from build123d import *

# Parameters (mm, degrees)
SKETCH1_W           = 40
SKETCH1_H           = 20
BOSS_EXTRUDE1_DEPTH = 4
M8_TAPPED_HOLE1_D   = 6.8
CUT_EXTRUDE1_DEPTH  = 4
CHAMFER1_SIZE       = 3
CHAMFER2_SIZE       = 0.5


with BuildPart() as part:
    # Sketch1 → Boss-Extrude1 (new body)
    with BuildSketch(Plane.XY):
        Rectangle(SKETCH1_W, SKETCH1_H)
    extrude(amount=BOSS_EXTRUDE1_DEPTH)

    # M8 Tapped Hole1 (through all)
    with Locations(Plane.XY.offset(4)):
        with Locations((-12.5, 0)):
            Hole(M8_TAPPED_HOLE1_D / 2)

    # Sketch4 → Cut-Extrude1 (cut)
    with BuildSketch(Plane.XY.offset(4)):
        with BuildLine():
            Line((7, 2.25), (17, 2.25))
            ThreePointArc((17, 2.25), (19.25, 0), (17, -2.25))
            Line((17, -2.25), (7, -2.25))
            ThreePointArc((7, -2.25), (4.75, 0), (7, 2.25))
        make_face()
    extrude(amount=-CUT_EXTRUDE1_DEPTH, mode=Mode.SUBTRACT)

    # Chamfer1
    chamfer1_edges = [part.edges().sort_by_distance(p)[0] for p in [
        (20, -10, 2),
        (-20, -10, 2),
        (-20, 10, 2),
        (20, 10, 2),
    ]]
    chamfer(chamfer1_edges, length=CHAMFER1_SIZE)

    # Chamfer2
    chamfer2_edges = [part.edges().sort_by_distance(p)[0] for p in [
        (20, 0, 0),
        (20, 0, 4),
        (0, -10, 0),
        (-20, 0, 0),
        (0, 10, 0),
        (0, -10, 4),
        (0, 10, 4),
        (-20, 0, 4),
    ]]
    chamfer(chamfer2_edges, length=CHAMFER2_SIZE)


solid = part.part
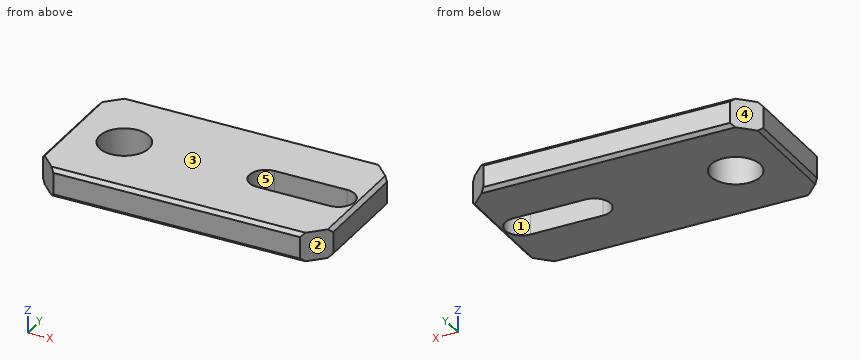
Source: CAD feature listing. Evaluate the final solid. Frame: model axes, mm. Face numbers are marked on the shaded views. A direction names the side the tool comes from. Give positions to 0.01 mm unless a question says otherwise; leave off trailing zeros. Loops run counter-clockwise (first coordinate to the right, second up) from the corner with the lowest first, then second, coordinate; pieces in that order, holes last. Notation, with made-up numbers: (42.25, 74) -> (66.25, 74) arc R24 ccw to (66.25, 84) -> close; hole circle Ø7 at (-9, 20). An arc over 180 degrees is marked (long way). Use a Markdown table: item, result. Add a question column.
1) Section query D-D, the plane x = 16.5. Return the cut outline in (y, z), then the cut area to 3 significant figures.
2) Pull-direction query (X, two-part tool) for the marked faces 3, 4 and 5; classes: +X half, -X half, draft (parallel to the pull), parting line (faces both ways), or undercut.
3) Reachability of the marked faces 1 and 2 from +Z, -Z, +X, -X, +Y, -Y: full face, straight path, thin tool, end or side. Return the list, or none.
4) Line query: line 1 along Y through (x, z) = (-12.5, 1.45); line 2 along X through (y, z) = (-2, 2.75); line 3 along X through (y, z) = (1, 0.55). Output: solid intervals per line, ascending. Write a range as [from, to].
5) Section query A-A, the plane y = 0. Return the cut outline in (x, z).
6) Section query B-B, the plane x = -12.5. Return the cut outline in (y, z).
7) Section query C-C, the plane z = 0.95. Return the cut outline in (x, y).
Numbers:
| question | item | result |
|---|---|---|
| 1 | outline | (-10, 0.5) -> (-9.5, 0) -> (-2.25, 0) -> (-2.25, 4) -> (-9.5, 4) -> (-10, 3.5) -> close; (2.25, 0) -> (9.5, 0) -> (10, 0.5) -> (10, 3.5) -> (9.5, 4) -> (2.25, 4) -> close |
| 1 | area | 61.5 mm2 |
| 2 | face 3 | draft |
| 2 | face 4 | -X half |
| 2 | face 5 | undercut |
| 3 | face 1 | +Z, -Z |
| 3 | face 2 | +Z, -Z, +X, -Y |
| 4 | line 1 | y = [-10, -3.4], [3.4, 10] |
| 4 | line 2 | x = [-20, -15.25], [-9.75, 5.97], [18.03, 20] |
| 4 | line 3 | x = [-20, -15.75], [-9.25, 4.98], [19.02, 20] |
| 5 | outline | (-20, 0.5) -> (-19.5, 0) -> (-15.9, 0) -> (-15.9, 4) -> (-19.5, 4) -> (-20, 3.5) -> close; (-9.1, 0) -> (4.75, 0) -> (4.75, 4) -> (-9.1, 4) -> close; (19.25, 0) -> (19.5, 0) -> (20, 0.5) -> (20, 3.5) -> (19.5, 4) -> (19.25, 4) -> close |
| 6 | outline | (-10, 0.5) -> (-9.5, 0) -> (-3.4, 0) -> (-3.4, 4) -> (-9.5, 4) -> (-10, 3.5) -> close; (3.4, 0) -> (9.5, 0) -> (10, 0.5) -> (10, 3.5) -> (9.5, 4) -> (3.4, 4) -> close |
| 7 | outline | (-20, -7) -> (-17, -10) -> (17, -10) -> (20, -7) -> (20, 7) -> (17, 10) -> (-17, 10) -> (-20, 7) -> close; hole circle Ø6.8 at (-12.5, 0); hole (7, -2.25) -> (17, -2.25) arc R2.25 ccw to (17, 2.25) -> (7, 2.25) arc R2.25 ccw to start |
